Source: CAD feature listing. Evaluate the final solid. Frame: model axes, mm. Round coordinates to 2 decimals unless told otherwise and drop trailing zeros. Loops run counter-clockwise (first coordinate to the right, second up) from the corner with the lowest first, then second, coordinate; pieces in that order, holes last. Notation, with made-up numbers: M -21,12.5 L 24,12.5 A25 ccw 24,42.5 Z; hole C 77,44 d5. An arc over 180 degrees is marked long. Answer as a JSON object with one key per item and string values.
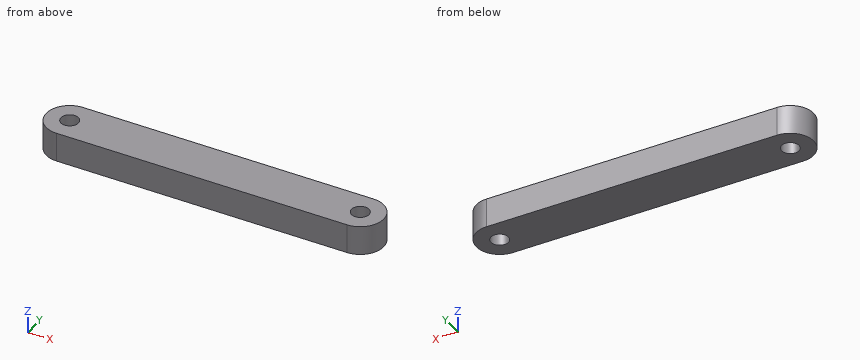
from build123d import *

# Parameters (mm, degrees)
BOSS_EXTRUDE1_DEPTH = 5
SKETCH3_R           = 1.5
CUT_EXTRUDE1_DEPTH  = 30.69848481


with BuildPart() as part:
    # Sketch1 → Boss-Extrude1 (new body)
    with BuildSketch(Plane.XY):
        with BuildLine():
            Line((-25, 4), (25, 4))
            ThreePointArc((25, 4), (29, 0), (25, -4))
            Line((25, -4), (-25, -4))
            ThreePointArc((-25, -4), (-29, 0), (-25, 4))
        make_face()
    extrude(amount=BOSS_EXTRUDE1_DEPTH)

    # Sketch3 → Cut-Extrude1 (cut, through all)
    with BuildSketch(Plane.XY.offset(5)):
        with Locations((-25, 0)):
            Circle(SKETCH3_R)
        with Locations((25, 0)):
            Circle(SKETCH3_R)
    extrude(amount=-CUT_EXTRUDE1_DEPTH, mode=Mode.SUBTRACT)


solid = part.part
Item 1: Section C-C on z = 2.85. Return the cut outline in (x, y).
Answer sheet:
{"outline": "M -25,-4 L 25,-4 A4 ccw 25,4 L -25,4 A4 ccw Z; hole C -25,0 d3; hole C 25,0 d3"}
Item 2: Section D-D on y = -2.5. Return the cut outline in (x, z).
Answer sheet:
{"outline": "M -28.12,0 L 28.12,0 L 28.12,5 L -28.12,5 Z"}
Item 3: Section B-B on x = -24. Return the cut outline in (y, z).
Answer sheet:
{"outline": "M -4,0 L -1.12,0 L -1.12,5 L -4,5 Z; M 1.12,0 L 4,0 L 4,5 L 1.12,5 Z"}
Item 4: Contact query for a flat-ended pin moving along its axis: pin 1 Ø2.5 at (x, y) = (-25, 0) entering from -Z. Output: stop coordinate, or through.
Answer sheet:
{"pin 1": "passes through"}
Item 5: Line query: probe 1 along Y at (x, z) = (-25, 2.8); probe 2 along X at (y, z) = (-0.25, 2.5); probe 3 along X at (y, z) = (-3, 0.95). Output: solid intervals per line, ascending. Write a range as from..to.
Answer sheet:
{"probe 1": "y = -4..-1.5, 1.5..4", "probe 2": "x = -28.99..-26.48, -23.52..23.52, 26.48..28.99", "probe 3": "x = -27.65..27.65"}
Item 6: Section A-A on y = 0. Return the cut outline in (x, z), then the cut area to 3 significant figures.
Answer sheet:
{"outline": "M -29,0 L -26.5,0 L -26.5,5 L -29,5 Z; M -23.5,0 L 23.5,0 L 23.5,5 L -23.5,5 Z; M 26.5,0 L 29,0 L 29,5 L 26.5,5 Z", "area": "260 mm²"}
